Build history of the part. All positions in model axes, mm. A direction names the side the tool comes from. Round coordinates to 2 decimals unless told otherwise and drop trailing zeros. Order: outer loops, then holes, each group sorted by start corner. A loop starts at its lowest first (then second) coordinate and runs counter-clockwise, first axis right, second up. Notation, with made-up numbers: (-30.75, 48.25) -> (5.25, 48.25) arc R22 cw to (5.25, 70.25) -> close; hole circle Ø6 at (-26, 35). An arc over 180 degrees is marked (long way). Answer as CSV lines item,"result". Start each with the question number.
```python
from build123d import *

# Parameters (mm, degrees)
CHAMFER_1_SIZE      = 1
FILLET_1_R          = 1
CHAMFER_3_SIZE      = 1.5
CUT_EXTRUDE_START   = 8
CUT_EXTRUDE_5_DEPTH = 8


with BuildPart() as part:
    # 草图1 → 旋转1 (revolve)
    with BuildSketch(Plane.XY, mode=Mode.PRIVATE) as revolve_1_sk:
        Polygon((0, 0), (0, 16), (7, 16), (7, 11.5), (9, 11.5), (9, 12), (22.252522581, 12), (25, 11), (69, 11), (69, 0), align=None)
    revolve(revolve_1_sk.sketch.rotate(Axis((-47.69348659, 0, 0), (1, 0, 0)), 90), axis=Axis((-47.69348659, 0, 0), (1, 0, 0)))

    # 倒角1
    chamfer_1_edges = [part.edges().sort_by_distance(p)[0] for p in [
        (0, 0, -16),
    ]]
    chamfer(chamfer_1_edges, length=CHAMFER_1_SIZE)

    # 圆角1
    fillet_1_edges = [part.edges().sort_by_distance(p)[0] for p in [
        (7, 0, -11.5),
    ]]
    fillet(fillet_1_edges, radius=FILLET_1_R)

    # 倒角3
    chamfer_3_edges = [part.edges().sort_by_distance(p)[0] for p in [
        (69, 0, -11),
    ]]
    chamfer(chamfer_3_edges, length=CHAMFER_3_SIZE)

    # 草图2 → 切除-拉伸5 (cut)
    with BuildSketch(Plane(origin=(0, 0, 0), x_dir=(0, 0, -1), z_dir=(1, 0, 0)).offset(CUT_EXTRUDE_START)):
        with BuildLine():
            Line((-10.583005244, 12), (10.583005244, 12))
            ThreePointArc((10.583005244, 12), (0, 16), (-10.583005244, 12))
        make_face()
    extrude(amount=-CUT_EXTRUDE_5_DEPTH, mode=Mode.SUBTRACT)


solid = part.part
```
Q1. Flat gauge pins, fed straight in: pin 1 Ø2 at (y, z) = (-3.5, 11) entering from +X; pin 2 Ø1 at (x, z) = (35, 3) entering from +Y; pin 3 Ø4 at (x, z) = (60.5, -11) entering from +Y; pin 4 Ø10 at (x, z) = (12.5, -1) entering from +Y. Where does each tip first touch, or does it go through?
Q2. Slice it at A-A, the plane z = 0. Write the cut outline in (x, y), plus the area to 3 significant figures.
Q3. Which spindle directions (+Z, -Z, +X, -X, +Y, -Y) get a long thin tool onto all of the face, cutting with end or side? Do faces 1 (the face through (7, -12.44, -2.45)), 2 (the face through (0, -2, 0)), 3 (the face through (8.5, -11.4, -1.5)). Say none if no direction does.
Q4. Probe L1, parallel to Y at x = 36.5, z = -3; L2, parallel to X at y = -7.75, z = 11; L3, parallel to Y at x = 26, z = -9. List the from-to ranges inside material, lowest first.
Q5. Slice it at C-C, the plane x = 51. Write the cut outline in (y, z), plus the area to 3 significant figures.
Q6. Slice it at B-B, the plane y = 0. Write the cut outline in (x, z).
Q7. Two-plate mould, pull along X, no slides. Class faces 4 (the face through (9, 10, -6)), 5 (the face through (46.55, 10.74, -2.38)), 6 (the face through (69, 0, 0)): +X half, -X half, draft (parallel to the pull), parting line (faces both ways), or undercut.
Solutions:
1,pin 1,"stops at x = 67.96"
1,pin 2,"stops at y = 10.71"
1,pin 3,"stops at y = 6.32"
1,pin 4,"stops at y = 12"
2,outline,"(0, -15) -> (1, -16) -> (7, -16) -> (7, -12.5) arc R1 cw to (8, -11.5) -> (9, -11.5) -> (9, -12) -> (22.25, -12) -> (25, -11) -> (67.5, -11) -> (69, -9.5) -> (69, 9.5) -> (67.5, 11) -> (25, 11) -> (22.25, 12) -> (9, 12) -> (9, 11.5) -> (8, 11.5) arc R1 cw to (7.13, 12) -> (0, 12) -> close"
2,area,"1,590 mm2"
3,face 1,"+X"
3,face 2,"+Z, -Z, -X, +Y, -Y"
3,face 3,"none"
4,L1,"y = -10.58 to 10.58"
4,L2,"x = 0 to 7"
4,L3,"y = -6.32 to 6.32"
5,outline,"circle Ø22 at (0, 0)"
5,area,"380 mm2"
6,outline,"(0, -15) -> (1, -16) -> (7, -16) -> (7, -12.5) arc R1 cw to (8, -11.5) -> (9, -11.5) -> (9, -12) -> (22.25, -12) -> (25, -11) -> (67.5, -11) -> (69, -9.5) -> (69, 9.5) -> (67.5, 11) -> (25, 11) -> (22.25, 12) -> (9, 12) -> (9, 11.5) -> (8, 11.5) arc R1 cw to (7, 12.5) -> (7, 16) -> (1, 16) -> (0, 15) -> close"
7,face 4,"undercut"
7,face 5,"draft"
7,face 6,"+X half"
